Build history of the part. All positions in model axes, mm. Face numbers are marked on the shaded views. A direction names the side the tool comes from. Round coordinates to 2 decimals unless told otherwise and drop trailing zeros. Write each loop counter-clockwise with the first axis right and the second up, starting at its lowest first coordinate (ties: lowest second). Pieces come first, ordered by that corner, then holes. Notation, with made-up numbers: (64, 66.5) -> (110, 66.5) arc R10 ccw to (110, 73.5) -> close; hole circle Ø1 at (-35, 87). An arc over 180 degrees is marked (long way). Answer as CSV lines item,"result".
from build123d import *

# Parameters (mm, degrees)
SKETCH_1_R          = 11
SKETCH_1_R_2        = 6
EXTRUDE_1_DEPTH     = 34
SKETCH_2_R          = 14
SKETCH_2_R_2        = 7
EXTRUDE_2_DEPTH     = 3
SKETCH_3_R          = 12.01734277
SKETCH_3_R_2        = 10
CUT_EXTRUDE_1_DEPTH = 15.5
SKETCH_4_W          = 13.23621111
SKETCH_4_H          = 1.977552999
CUT_EXTRUDE_2_DEPTH = 32
CUT_EXTRUDE_3_DEPTH = 42.964270517
SKETCH_6_W          = 1
SKETCH_6_H          = 1.2
EXTRUDE_START       = 2.7
SKETCH_7_R          = 10
EXTRUDE_3_DEPTH     = 2.7


with BuildPart() as part:
    # 草图1 → 凸台-拉伸1 (new body)
    with BuildSketch(Plane.XY):
        Circle(SKETCH_1_R)
        Circle(SKETCH_1_R_2, mode=Mode.SUBTRACT)
    extrude(amount=EXTRUDE_1_DEPTH)

    # 草图2 → 凸台-拉伸2 (add)
    with BuildSketch(Plane.XY.offset(34)):
        Circle(SKETCH_2_R)
        Circle(SKETCH_2_R_2, mode=Mode.SUBTRACT)
    extrude(amount=EXTRUDE_2_DEPTH)

    # 草图3 → 切除-拉伸1 (cut)
    with BuildSketch(Plane(origin=(0, 0, 0), x_dir=(-1, 0, 0), z_dir=(0, 0, -1))):
        Circle(SKETCH_3_R)
        Circle(SKETCH_3_R_2, mode=Mode.SUBTRACT)
    extrude(amount=-CUT_EXTRUDE_1_DEPTH, mode=Mode.SUBTRACT)

    # 草图4 → 切除-拉伸2 (cut)
    with BuildSketch(Plane(origin=(0, 0, 0), x_dir=(-1, 0, 0), z_dir=(0, 0, -1))):
        with Locations((1.1977553, 10.9887765)):
            Rectangle(SKETCH_4_W, SKETCH_4_H)
    extrude(amount=-CUT_EXTRUDE_2_DEPTH, mode=Mode.SUBTRACT)

    # 草图5 → 切除-拉伸3 (cut, through all)
    with BuildSketch(Plane.XY.offset(37)):
        Polygon((7, -4.041451884), (7, 4.041451884), (0, 8.082903769), (-7, 4.041451884), (-7, -4.041451884), (0, -8.082903769), align=None)
    extrude(amount=-CUT_EXTRUDE_3_DEPTH, mode=Mode.SUBTRACT)

    # 草图6 → 切除-旋转1 (revolve, cut)
    with BuildSketch(Plane(origin=(0, 0, 0), x_dir=(1, 0, 0), z_dir=(0, 1, 0)), mode=Mode.PRIVATE) as cut_revolve_1_sk:
        with Locations((10, -2.9)):
            Rectangle(SKETCH_6_W, SKETCH_6_H)
    revolve(cut_revolve_1_sk.sketch.rotate(Axis((0, 0, -1.695132032), (0, 0, 1)), 180), axis=Axis((0, 0, -1.695132032), (0, 0, 1)), mode=Mode.SUBTRACT)

    # 草图7 → 凸台-拉伸3 (add)
    with BuildSketch(Plane(origin=(0, 0, 0), x_dir=(-1, 0, 0), z_dir=(0, 0, -1)).offset(EXTRUDE_START)):
        Circle(SKETCH_7_R)
        Polygon((7, -4.041451884), (7, 4.041451884), (0, 8.082903769), (-7, 4.041451884), (-7, -4.041451884), (0, -8.082903769), align=None, mode=Mode.SUBTRACT)
    extrude(amount=-EXTRUDE_3_DEPTH)


solid = part.part
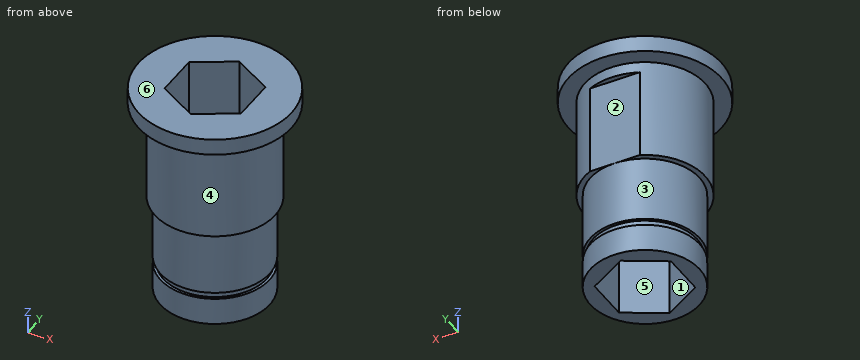
1. Cut at A-A, the plane z = 1.5. Write the cut outline in (x, y).
Results found:
outline,"circle Ø20 at (0, 0); hole (-7, -4.04) -> (0, -8.08) -> (7, -4.04) -> (7, 4.04) -> (0, 8.08) -> (-7, 4.04) -> close"
2. Mould opens along X. For the marked faces 4, 5 and 6 say: +X half, -X half, draft (parallel to the pull), parting line (faces both ways), or undercut.
Results found:
face 4,"parting line"
face 5,"undercut"
face 6,"draft"
3. Cut at D-D, the plane z = 32.5. Write the cut outline in (x, y).
Results found:
outline,"circle Ø22 at (0, 0); hole (-7, -4.04) -> (0, -8.08) -> (7, -4.04) -> (7, 4.04) -> (0, 8.08) -> (-7, 4.04) -> close"
4. Drop flat-ended pins along their axis: pin 1 Ø5 at (y, z) = (4.5, 25.5) entering from +X; pin 2 Ø12 at (x, z) = (-3.5, 27) entering from -Y; pin 3 Ø1.1 at (x, y) = (-1.5, 10.5) entering from -Z. Give the stop position or say it passes through.
Results found:
pin 1,"stops at x = 10.82"
pin 2,"stops at y = -11"
pin 3,"stops at z = 15.5"
5. Probe line 1 along X through (y, z) = (0, 8.5); line 2 along Z through (x, y) = (8.5, -7.25); line 3 along Y through (x, z) = (0, 25.5). List the from-to ranges inside material, lowest first.
Results found:
line 1,"x = -10 to -7, 7 to 10"
line 2,"z = 34 to 37"
line 3,"y = -11 to -8.08, 8.08 to 10"
6. Which spindle directions (+Z, -Z, +X, -X, +Y, -Y) get a long thin tool onto all of the face, cutting with end or side? Do the marked faces 1, 2 and 3. Say none if no direction does.
Results found:
face 1,"+Z, -Z"
face 2,"-Z, +X, -X, +Y"
face 3,"-Z"
7. Cut at B-B, the plane y = 0. Write the cut outline in (x, z), then the cut area to 3 significant figures.
Results found:
outline,"(-14, 34) -> (-11, 34) -> (-11, 15.5) -> (-10, 15.5) -> (-10, 3.5) -> (-9.5, 3.5) -> (-9.5, 2.3) -> (-10, 2.3) -> (-10, -2.7) -> (-7, -2.7) -> (-7, 37) -> (-14, 37) -> close; (7, -2.7) -> (10, -2.7) -> (10, 2.3) -> (9.5, 2.3) -> (9.5, 3.5) -> (10, 3.5) -> (10, 15.5) -> (11, 15.5) -> (11, 34) -> (14, 34) -> (14, 37) -> (7, 37) -> close"
area,"298 mm2"
8. Cut at C-C, the plane x = -2.25. Write the cut outline in (y, z), then the cut area to 3 significant figures.
Results found:
outline,"(-13.82, 34) -> (-10.77, 34) -> (-10.77, 15.5) -> (-9.74, 15.5) -> (-9.74, 3.5) -> (-9.23, 3.5) -> (-9.23, 2.3) -> (-9.74, 2.3) -> (-9.74, -2.7) -> (-6.78, -2.7) -> (-6.78, 37) -> (-13.82, 37) -> close; (6.78, -2.7) -> (9.74, -2.7) -> (9.74, 2.3) -> (9.23, 2.3) -> (9.23, 3.5) -> (9.74, 3.5) -> (9.74, 15.5) -> (10, 15.5) -> (10, 32) -> (10.77, 32) -> (10.77, 34) -> (13.82, 34) -> (13.82, 37) -> (6.78, 37) -> close"
area,"283 mm2"
